Build history of the part. All positions in model axes, mm. Face numbers are marked on the shaded views. A direction names the side the tool comes from. Give positions to 0.01 mm unless a question says otherwise; leave off trailing zeros. Loops run counter-clockwise (first coordinate to the right, second up) from the corner with the lowest first, then second, coordinate; pieces in that order, holes last. Notation, with made-up numbers: M -20,-24.75 L 29,-24.75 A6 cw 29,-18.75 Z; hole C 4,69 d3. An arc over 180 degrees is marked long. Answer as a JSON object with one key per item and string values. Group by question number.
1. Slice it at A-A (z = 0). List the corners of the cut face in (x, y), then the cut area to 3 significant figures.
2. 3-axis set-ups, long thin cutter, end or side, ignore diameter. For the marked faces 1, 2 and 3: which of +Z, -Z, +X, -X, +Y, -Y reach the whole face in a straight line?
3. Slice it at B-B (x = 0). List the corners of the cut face in (y, z).
4. Slice it at D-D (y = 31). List the corners of the cut face in (x, z), then the cut area to 3 significant figures.
5. Drill centre lines: line 1 along Y through (x, z) = (-7.5, -36.5); line 2 along Z through (x, y) = (-1.5, 140.5); line 3 along Z through (x, y) = (24.5, 55) (3 decimals). Where is each one in solid material? Low to high. Write a range as [from, to].
6. Slice it at C-C (y = 147.5). List the corners of the cut face in (x, z), then the cut area to 3 significant figures.
7. Drop flat-ended pins along their axis: pin 1 Ø3 at (x, y) = (20.5, 62.5) entering from -Z; pin 2 Ø8 at (x, y) = (-32.5, 34) entering from +Z; pin 3 Ø3 at (x, z) = (10, -37.5) entering from -Y. Give the stop position or say it passes through.
from build123d import *

# Parameters (mm, degrees)
CUT_EXTRUDE1_DEPTH = 176.211301005


with BuildPart() as part:
    # Sketch1 → Revolve1 (revolve)
    with BuildSketch(Plane.XY):
        Polygon((0, 0), (-34, 0), (-35, 1), (-35, 28), (-55, 28), (-55, 53), (-35, 53), (-35, 209), (-34, 210), (0, 210), align=None)
    revolve(axis=Axis((0, 210, 0), (0, -1, 0)))

    # Sketch2 → Cut-Extrude1 (cut, through all)
    with BuildSketch(Plane(origin=(0, 53, 0), x_dir=(1, 0, 0), z_dir=(0, 1, 0))):
        with BuildLine():
            Line((-22.912878475, 50), (22.912878475, 50))
            ThreePointArc((22.912878475, 50), (0, 55), (-22.912878475, 50))
        make_face()
        with BuildLine():
            Line((-22.912878475, -50), (22.912878475, -50))
            ThreePointArc((22.912878475, -50), (0, -55), (-22.912878475, -50))
        make_face()
    extrude(amount=-CUT_EXTRUDE1_DEPTH, mode=Mode.SUBTRACT)


solid = part.part
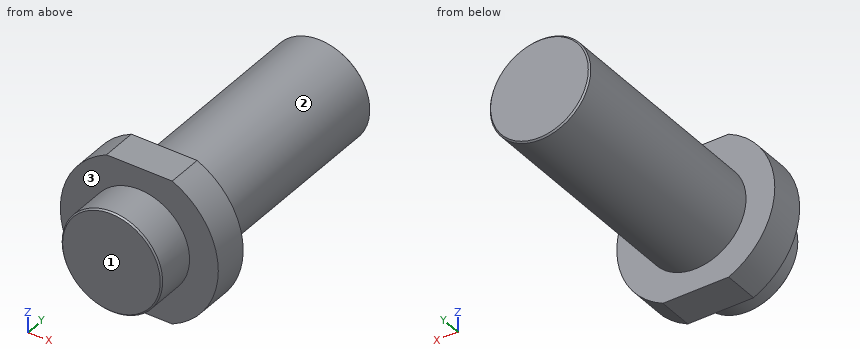
Established:
{
 "1": {"outline": "M -55,28 L -35,28 L -35,1 L -34,0 L 34,0 L 35,1 L 35,28 L 55,28 L 55,53 L 35,53 L 35,209 L 34,210 L -34,210 L -35,209 L -35,53 L -55,53 Z", "area": "15,700 mm^2"},
 "2": {"face 1": "+Z, -Z, +X, -X, -Y", "face 2": "+Y", "face 3": "-Y"},
 "3": {"outline": "M 0,-34 L 1,-35 L 28,-35 L 28,-50 L 53,-50 L 53,-35 L 209,-35 L 210,-34 L 210,34 L 209,35 L 53,35 L 53,50 L 28,50 L 28,35 L 1,35 L 0,34 Z"},
 "4": {"outline": "M -22.91,-50 L 22.91,-50 A55 ccw 22.91,50 L -22.91,50 A55 ccw Z", "area": "9,190 mm^2"},
 "5": {"line 1": "y = [28, 53]", "line 2": "z = [-34.97, 34.97]", "line 3": "z = [-24.995, 24.995]"},
 "6": {"outline": "C 0,0 d70", "area": "3,850 mm^2"},
 "7": {"pin 1": "stops at z = -29.39", "pin 2": "stops at z = 47.04", "pin 3": "stops at y = 28"}
}
